from build123d import *

# Parameters (mm, degrees)
SKETCH1_R              = 140
BOSS_EXTRUDE1_DEPTH    = 120
SKETCH3_R              = 10
CUT_EXTRUDE1_DEPTH     = 1
M10_TAPPED_HOLE1_D     = 8.5
M10_TAPPED_HOLE1_DEPTH = 40
M10_TAPPED_HOLE1_TIP   = 2.553657631
SKETCH7_R              = 11
CUT_EXTRUDE2_DEPTH     = 11303.32306496
FILLET1_R              = 3
CIRPATTERN1_COUNT      = 6
M16_TAPPED_HOLE2_D     = 14
M16_TAPPED_HOLE2_DEPTH = 38
M16_TAPPED_HOLE2_TIP   = 4.206024333


with BuildPart() as part:
    # Sketch1 → Boss-Extrude1 (new body)
    with BuildSketch(Plane.XY):
        with BuildLine():
            Line((10876.867117242, -355.960833708), (10876.867117242, -495.960833708))
            ThreePointArc((10876.867117242, -495.960833708), (10873.938185054, -503.03190152), (10866.867117242, -505.960833708))
            Line((10866.867117242, -505.960833708), (10816.867117242, -505.960833708))
            Line((10816.867117242, -505.960833708), (10816.867117242, -545.960833708))
            Line((10816.867117242, -545.960833708), (11296.867117242, -545.960833708))
            Line((11296.867117242, -545.960833708), (11296.867117242, -505.960833708))
            Line((11296.867117242, -505.960833708), (11246.867117242, -505.960833708))
            ThreePointArc((11246.867117242, -505.960833708), (11239.796049431, -503.03190152), (11236.867117242, -495.960833708))
            Line((11236.867117242, -495.960833708), (11236.867117242, -355.960833708))
            ThreePointArc((11236.867117242, -355.960833708), (11056.867117242, -175.960833708), (10876.867117242, -355.960833708))
        make_face()
        with Locations((11056.867117242, -355.960833708)):
            Circle(SKETCH1_R, mode=Mode.SUBTRACT)
    extrude(amount=BOSS_EXTRUDE1_DEPTH)

    # Sketch3 → Cut-Extrude1 (cut)
    with BuildSketch(Plane(origin=(0, -175.960833708, 0), x_dir=(1, 0, 0), z_dir=(0, 1, 0))):
        with Locations(Location((11056.867117242, -60, 0), (0, 0, 270))):
            Circle(SKETCH3_R)
    extrude(amount=-CUT_EXTRUDE1_DEPTH, mode=Mode.SUBTRACT)

    # M10 Tapped Hole1
    with Locations(Plane(origin=(0, -176.960833708, 0), x_dir=(1, 0, 0), z_dir=(0, 1, 0))):
        with Locations((11056.867117242, -60)):
            Hole(M10_TAPPED_HOLE1_D / 2, depth=M10_TAPPED_HOLE1_DEPTH)
            with Locations((0, 0, -(M10_TAPPED_HOLE1_DEPTH + M10_TAPPED_HOLE1_TIP / 2))):  # 118° drill point
                Cone(0, M10_TAPPED_HOLE1_D / 2, M10_TAPPED_HOLE1_TIP, mode=Mode.SUBTRACT)

    # Sketch7 → Cut-Extrude2 (cut, through all)
    with BuildSketch(Plane(origin=(0, -505.960833708, 0), x_dir=(1, 0, 0), z_dir=(0, 1, 0))):
        with Locations(Location((10836.867117242, -20, 0), (0, 0, 270))):
            Circle(SKETCH7_R)
        with Locations(Location((10836.867117242, -100, 0), (0, 0, 270))):
            Circle(SKETCH7_R)
        with Locations(Location((11276.867117242, -100, 0), (0, 0, 90))):
            Circle(SKETCH7_R)
        with Locations(Location((11276.867117242, -20, 0), (0, 0, 90))):
            Circle(SKETCH7_R)
    extrude(amount=-CUT_EXTRUDE2_DEPTH, mode=Mode.SUBTRACT)

    # Fillet1
    fillet1_edges = [part.edges().sort_by_distance(p)[0] for p in [
        (11296.867117242, -505.960833708, 60),
        (10816.867117242, -505.960833708, 60),
    ]]
    fillet(fillet1_edges, radius=FILLET1_R)

    # Sketch9 → M16 Tapped Hole1 (revolve, cut)
    with BuildSketch(Plane(origin=(10975.617117242, -215.231705593, 120), x_dir=(0, -1, 0), z_dir=(1, 0, 0))):
        Polygon((0, 0), (0, 42.206024333), (7, 38), (7, 0), align=None)
    m16_tapped_hole1 = revolve(axis=Axis((10975.617117242, -215.231705593, 126.35), (0, 0, -1)), mode=Mode.SUBTRACT)

    # CirPattern1: M16 Tapped Hole1 ×6 about axis
    cirpattern1_axis = Axis((11056.867117242, -355.960833708, 0), (0, 0, 1))
    for i in range(1, CIRPATTERN1_COUNT):
        add(m16_tapped_hole1.rotate(cirpattern1_axis, i * 360 / CIRPATTERN1_COUNT), mode=Mode.SUBTRACT)

    # M16 Tapped Hole2
    with Locations(Plane(origin=(0, 0, 0), x_dir=(-1, 0, 0), z_dir=(0, 0, -1))):
        with Locations((-11138.117117242, -215.231705593), (-10975.617117242, -215.231705593), (-10894.367117242, -355.960833708), (-10975.617117242, -496.689961823), (-11138.117117242, -496.689961823), (-11219.367117242, -355.960833708)):
            Hole(M16_TAPPED_HOLE2_D / 2, depth=M16_TAPPED_HOLE2_DEPTH)
            with Locations((0, 0, -(M16_TAPPED_HOLE2_DEPTH + M16_TAPPED_HOLE2_TIP / 2))):  # 118° drill point
                Cone(0, M16_TAPPED_HOLE2_D / 2, M16_TAPPED_HOLE2_TIP, mode=Mode.SUBTRACT)


solid = part.part
Verification items for the finished model (mm, model axes). A direction names the side the tool comes from. Give positions to 0.01 mm unless a question says otherwise; leave off trailing zeros. Loops run counter-clockwise (first coordinate to the right, second up) from the corner with the lowest first, then second, coordinate; pieces in that order, holes last. Notation, with made-up numbers: (31, -15.5) - (84, -15.5) arc R22 cw to (84, 4.5) - close; hole circle Ø6 at (82.5, 42.25). An arc over 180 degrees is marked (long way). Write item = value, one per line. Start each with the question number.
Q1. Tool access check on faces 5 (the face through (11060.825, -176.004, 45.827)), 6 (the face through (11236.867, -427, 59)), 7 (the face through (10981.83, -218.46, 101.27)), 8 (the face through (10982.083, -217.913, 19.266)). Record the directions out of +Z, -Z, +X, -X, +Y, -Y that give a thin tool (end or side, any length) a straight path to the whole face; none if there is none.
Q2. Cross-section at B-B, the plane y = -403.5. Enter the section's corners in (x, z).
Q3. Thickness scan on line 1 (X direction, y = -528, z = 20); line 2 (Y direction, x = 11062, z = 61.5); line 3 (Y direction, x = 10952.5, z = 13.5). Record the ranges inside material, lowest first.
Q4. Cross-section at C-C, the plane x = 11175. Enter the section's corners in (y, z), and give its area (3 significant figures).
Q5. Mould release check, pull along Z, two halves, no side actions. Record for faces 1 (the face through (11271, -505.961, 59)), 2 (the face through (11136.93, -496.953, 78.524)), 3 (the face through (11055, -176.961, 64)), 4 (the face through (11136.994, -215.697, 41.476)): released by +Z, released by -Z, zero draft, split by the parting line, or undercut.
Q6. Cross-section at A-A, the plane z = 20. State how many separate pieces and enclosed holes the cut face has, and give its area (3 significant figures).
Q7. Cross-section at D-D, the plane y = -514. Enter the section's corners in (x, z), and give its area (3 significant figures).
Q8. Depth check by flat-ended pin: P1, Ø1, axis at y = -285.5, z = 102.5, coming from the -X side; P2, Ø1, axis at y = -437.5, z = 55, coming from the -X side; P3, Ø4, axis at x = 11068, y = -218, coming from the +Z side; P4, Ø12.5, axis at x = 10975.62, y = -496.69, coming from the +Z side. Enter the tip coordinate at first touch or a pass-through.
Answer key:
q1.face_5 = +Z, -Z, +Y
q1.face_6 = +Z, -Z, +X, +Y
q1.face_7 = +Z
q1.face_8 = -Z
q2.outline = (10876.87, 0) - (10925.19, 0) - (10925.19, 120) - (10876.87, 120) - close; (11188.55, 0) - (11236.87, 0) - (11236.87, 120) - (11188.55, 120) - close
q3.line_1 = 10816.87 to 10825.87, 10847.87 to 11265.87, 11287.87 to 11296.87
q3.line_2 = -545.96 to -495.87, -216.05 to -176.96
q3.line_3 = -545.96 to -449.27, -262.65 to -209.31
q4.outline = (-545.96, 0) - (-431.09, 0) - (-431.09, 120) - (-545.96, 120) - close; (-280.83, 0) - (-220.15, 0) - (-220.15, 120) - (-280.83, 120) - close
q4.area = 21,100 mm^2
q5.face_1 = zero draft
q5.face_2 = released by +Z
q5.face_3 = undercut
q5.face_4 = released by -Z
q6.separate_pieces = 3
q6.enclosed_holes = 7
q6.area = 59,900 mm^2
q7.outline = (10816.87, 0) - (11296.87, 0) - (11296.87, 120) - (10816.87, 120) - close; hole circle Ø22 at (10836.87, 20); hole circle Ø22 at (10836.87, 100); hole circle Ø22 at (11276.87, 20); hole circle Ø22 at (11276.87, 100)
q7.area = 56,100 mm^2
q8.P1 = 10891.02
q8.P2 = 10876.87
q8.P3 = 120
q8.P4 = 81.55
